```python
from build123d import *

# Parameters (mm, degrees)
EXTRUDE_1_DEPTH     = 510
SKETCH_2_R          = 2.25
CUT_EXTRUDE_1_DEPTH = 20


with BuildPart() as part:
    # 草图1 → 凸台-拉伸1 (new, symmetric)
    with BuildSketch(Plane.XY):
        Polygon((-37.5, 0), (-39.5, 0), (-39.5, 4.3), (-30, 6), (30, 6), (39.5, 4.3), (39.5, 0), (37.5, 0), (37.5, 2.122105263), (29.8, 3.5), (-29.8, 3.5), (-37.5, 2.122105263), align=None)
    extrude(amount=EXTRUDE_1_DEPTH, both=True)

    # 草图2 → 切除-拉伸1 (cut)
    with BuildSketch(Plane(origin=(0, 6, 0), x_dir=(1, 0, 0), z_dir=(0, 1, 0))):
        with Locations(Location((-20, 505, 0), (0, 0, 270))):
            Circle(SKETCH_2_R)
        with Locations(Location((20, 505, 0), (0, 0, 270))):
            Circle(SKETCH_2_R)
    cut_extrude_1 = extrude(amount=-CUT_EXTRUDE_1_DEPTH, mode=Mode.SUBTRACT)

    # 镜向1: 切除-拉伸1 across plane
    add(cut_extrude_1.mirror(Plane.XY), mode=Mode.SUBTRACT)


solid = part.part
```
Work out the finished part from the listing and answer in its coordinate system (mm). Coordinates: 2 decimals unless noted, no trailing zeros. Write each loop counter-clockwise with the first axis right and the second up, starting at its lowest first coordinate (ties: lowest second). Pieces come first, ordered by that corner, then holes.
Q1. A cutting plane is placed at C-C, the plane x = -9. Give the vertices of the cut face in (y, z).
Q2. Determine the mould class of faces 1 (the face through (0, 3.5, 7)), 2 (the face through (0, 6, 7)) for opening direction X: released by +X, released by -X, zero draft, split by the parting line, or undercut.
Q3. Each of these flat-tipped pins is pushed along its axis until it touches: pin 1 Ø1 at (x, z) = (5, 28.5) entering from -Y; pin 2 Ø4 at (x, z) = (-20, -505) entering from -Y. Where does it stop, or does it pass through?
Q4. Find the intervals of material crossed by line 1 (X direction, y = 4.15, z = -505); line 2 (X direction, y = 0.7, z = 79); line 3 (Z direction, x = 18.5, y = 5.6), in increasing order.
Q5. A cutting plane is placed at A-A, the plane y = 1.2. Give the vertices of the cut face in (x, z), then the cut area to 3 significant figures.
Q6. A cutting plane is placed at B-B, the plane z = 407. Give the vertices of the cut face in (x, y), then the cut area to 3 significant figures.
Findings below:
1. outline: (3.5, -510) - (6, -510) - (6, 510) - (3.5, 510) - close
2. face 1: undercut
2. face 2: zero draft
3. pin 1: stops at y = 3.5
3. pin 2: passes through
4. line 1: x = -39.5 to -22.25, -17.75 to 17.75, 22.25 to 39.5
4. line 2: x = -39.5 to -37.5, 37.5 to 39.5
4. line 3: z = -510 to -506.68, -503.32 to 503.32, 506.68 to 510
5. outline: (-39.5, -510) - (-37.5, -510) - (-37.5, 510) - (-39.5, 510) - close; (37.5, -510) - (39.5, -510) - (39.5, 510) - (37.5, 510) - close
5. area: 4,080 mm2
6. outline: (-39.5, 0) - (-37.5, 0) - (-37.5, 2.12) - (-29.8, 3.5) - (29.8, 3.5) - (37.5, 2.12) - (37.5, 0) - (39.5, 0) - (39.5, 4.3) - (30, 6) - (-30, 6) - (-39.5, 4.3) - close
6. area: 206 mm2
